from build123d import *

# Parameters (mm, degrees)
SKETCH_1_W              = 28
SKETCH_1_H              = 18
EXTRUDE_1_DEPTH         = 4
SKETCH_2_R              = 5
CUT_EXTRUDE_1_DEPTH     = 19.466185313
HOLE_WIZARD_M4_1_REACH  = 31.682
HOLE_WIZARD_M4_1_BORE_R = 1.65
HOLE_WIZARD_M4_2_D      = 3.3
HOLE_WIZARD_M4_3_D      = 3.3
CHAMFER_1_SIZE          = 1


with BuildPart() as part:
    # 草图1 → 凸台-拉伸1 (new, symmetric)
    with BuildSketch(Plane(origin=(0, 0, 0), x_dir=(0, 0, -1), z_dir=(1, 0, 0))):
        Rectangle(SKETCH_1_W, SKETCH_1_H)
    extrude(amount=EXTRUDE_1_DEPTH, both=True)

    # 草图2 → 切除-拉伸1 (cut, through all)
    with BuildSketch(Plane(origin=(4, 0, 0), x_dir=(0, 0, -1), z_dir=(1, 0, 0))):
        with Locations((-4, 0)):
            Circle(SKETCH_2_R)
    extrude(amount=-CUT_EXTRUDE_1_DEPTH, mode=Mode.SUBTRACT)

    # M4 螺纹孔1 bore → M4 螺纹孔1 (cut, up to next)
    with BuildSketch(Plane.XY.offset(14), mode=Mode.PRIVATE) as hole_wizard_m4_1_sk1:
        Circle(HOLE_WIZARD_M4_1_BORE_R)
    hole_wizard_m4_1_tool1 = extrude(hole_wizard_m4_1_sk1.sketch, amount=-HOLE_WIZARD_M4_1_REACH, mode=Mode.PRIVATE) & part.part
    add(hole_wizard_m4_1_tool1.solids().sort_by_distance((0, 0, 14))[0], mode=Mode.SUBTRACT)

    # M4 螺纹孔2 (through all)
    with Locations(Plane(origin=(4, 0, 0), x_dir=(0, 0, -1), z_dir=(1, 0, 0))):
        with Locations((8.5, 0)):
            Hole(HOLE_WIZARD_M4_2_D / 2)

    # M4 螺纹孔3 (through all)
    with Locations(Plane(origin=(0, 9, 0), x_dir=(1, 0, 0), z_dir=(0, 1, 0))):
        with Locations((0, -4)):
            Hole(HOLE_WIZARD_M4_3_D / 2)

    # 倒角1
    chamfer_1_edges = [part.edges().sort_by_distance(p)[0] for p in [
        (0, 9, 14),
        (0, 9, -14),
        (0, -9, -14),
        (0, -9, 14),
    ]]
    chamfer(chamfer_1_edges, length=CHAMFER_1_SIZE)


solid = part.part
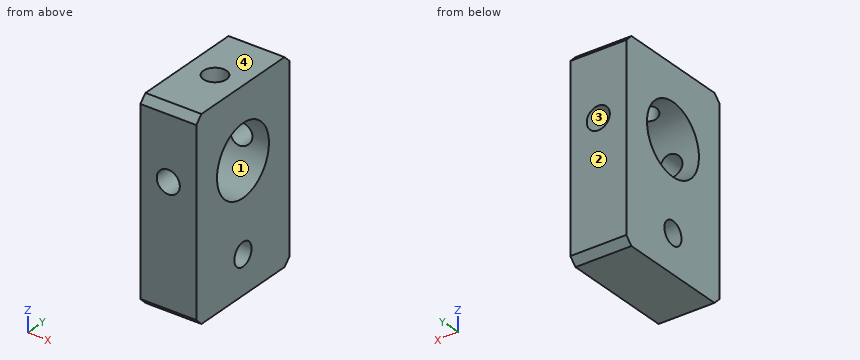
Part model, mm, in its own coordinate system. Face numbers are marked on the shaded views. Give positions to 0.01 mm unless a question says otherwise; leave off trailing zeros. Loops run counter-clockwise (first coordinate to the right, second up) from the corner with the lowest first, then second, coordinate; pieces in that order, holes last. Notation, with made-up numbers: M -22,-37.75 L 24,-37.75 A27 cw 24,-12.75 Z; hole C -5.75,38 d3. An arc over 180 degrees is marked long. Put each result on its own line as item: value. Start each with the question number.
1) Saw through at C-C (z = -8.5). List the corners of the cut face in (x, y).
2) Probe probe 1 along Y at (x, z) = (-2.5, 4); probe 2 along Y at (x, z) = (-0.75, -8.5); probe 3 along Z at (x, y) = (0, -6.8). List the from-to ranges inside material, lowest first.
3) Saw through at B-B (x = 0). List the corners of the cut face in (y, z), then the cut area to 3 significant figures.
4) Saw through at D-D (y = 4.25). List the corners of the cut face in (x, z).
5) Flat gauge pin, fed straight in: pin 1 (2.5 mm diameter, centred on x = 0, y = 0, fed in from +Z). Where does the tip first touch, or does it go through?
6) Saw through at A-A (z = 4). List the corners of the cut face in (x, y).
7) Pull direction Z, two halves, no side cores. Call the marked faces 1, 2, 3 and 4: +Z half, -Z half, draft (parallel to the pull), parting line (faces both ways), or undercut.
Numbers:
1. outline: M -4,-9 L 4,-9 L 4,-1.65 L -4,-1.65 Z; M -4,1.65 L 4,1.65 L 4,9 L -4,9 Z
2. probe 1: -9 to -5, 5 to 9
2. probe 2: -9 to -1.65, 1.65 to 9
2. probe 3: -14 to 2.35, 5.65 to 14
3. outline: M -9,-13 L -8,-14 L 8,-14 L 9,-13 L 9,2.35 L 4.72,2.35 A5 cw -4.72,2.35 L -9,2.35 Z; M -9,5.65 L -4.72,5.65 A5 cw -1.65,8.72 L -1.65,14 L -8,14 L -9,13 Z; M 1.65,8.72 A5 cw 4.72,5.65 L 9,5.65 L 9,13 L 8,14 L 1.65,14 Z; hole C 0,-8.5 d3.3
3. area: 371 mm^2
4. outline: M -4,-14 L 4,-14 L 4,1.37 L -4,1.37 Z; M -4,6.63 L 4,6.63 L 4,14 L -4,14 Z
5. pin 1: z = -0.84
6. outline: M -4,-9 L -1.65,-9 L -1.65,-5 L -4,-5 Z; M -4,5 L -1.65,5 L -1.65,9 L -4,9 Z; M 1.65,-9 L 4,-9 L 4,-5 L 1.65,-5 Z; M 1.65,5 L 4,5 L 4,9 L 1.65,9 Z
7. face 1: undercut
7. face 2: draft
7. face 3: undercut
7. face 4: +Z half
